Build history of the part. All positions in model axes, mm. A direction names the side the tool comes from. Give positions to 0.01 mm unless a question says otherwise; leave off trailing zeros. Order: outer loops, then holes, each group sorted by start corner. A loop starts at its lowest first (then second) coordinate and runs counter-clockwise, first axis right, second up. Notation, with made-up numbers: (88, -19.75) - (109, -19.75) arc R19 cw to (109, 15.25) - close; hole circle Ø9 at (44.5, 7.25). An arc over 180 degrees is marked (long way). Write each question's results on one line, items separated by ' | '. Start each with the question number.
1) Two-plate mould, pull along X, no slides. Class faces 1 (the face through (23, 97, -5)), 2 (the face through (-22, 98, -5)), 3 (the face through (1.774, 32.783, -1.775)): +X half, -X half, draft (parallel to the pull), parting line (faces both ways), or undercut.
2) Cut at B-B on x = 0. State how many separate pieces and enclosed holes the cut face has, plus the area to 3 significant figures.
3) Drill centre lines: line 1 along Y through (x, z) = (0, -6.75); line 2 along Y through (x, z) = (0, -2.1); line 3 along Z through (x, y) = (12.5, 6.25). Where is each one in solid material? Low to high. Write a range as from..to.
4) Cut at A-A on y = 60. List the corners of the cut face in (x, z), plus the area to 3 significant figures.
5) Cut at D-D on x = 12.5. List the corners of the cut face in (y, z).
6) Tool access for faces 4 (the face through (25, 38, -9)), 5 (the face through (0.716, 35.453, -6.845)), 6 (the face through (0, 54, -10)): list every direction of +Z, -Z, +X, -X, +Y, -Y with a clear straight run to the whole face (end or side of a thin tool).
7) Drop flat-ended pins along their axis: pin 1 Ø25 at (x, y) = (-1, 68) entering from -Z; pin 2 Ø9 at (x, y) = (0, 60) entering from +Z; pin 3 Ø9 at (x, z) = (6.5, -20.5) entering from +Y; pin 4 Ø5.5 at (x, y) = (0, 90) entering from +Z. Give the stop position or say it passes through.
8) Cut at C-C on z = -25. List the corners of the cut face in (x, y).
from build123d import *

# Parameters (mm, degrees)
EXTRUDE_2_DEPTH              = 25
HOLE_WIZARD_6_5_6_5_1_D      = 6.5
HOLE_WIZARD_M6_1_D           = 6.6
HOLE_WIZARD_M6_1_CBORE_D     = 11
HOLE_WIZARD_M6_1_CBORE_DEPTH = 6.4
CHAMFER_1_SIZE               = 5


with BuildPart() as part:
    # 草图2 → 拉伸-薄壁2 (new, symmetric)
    with BuildSketch(Plane(origin=(0, 0, 0), x_dir=(0, 0, -1), z_dir=(1, 0, 0))):
        Polygon((0, 100), (0, 0), (40, 0), (40, 10), (10, 10), (10, 100), align=None)
    extrude(amount=EXTRUDE_2_DEPTH, both=True)

    # Ø6.5 (6.5) 直径孔1 (through all)
    with Locations(Plane(origin=(0, 10, 0), x_dir=(1, 0, 0), z_dir=(0, 1, 0))):
        with Locations((-12.5, 25), (12.5, 25)):
            Hole(HOLE_WIZARD_6_5_6_5_1_D / 2)

    # M6 六角凹头螺钉的柱形沉头孔1 (through all)
    with Locations(Plane(origin=(0, 0, -10), x_dir=(-1, 0, 0), z_dir=(0, 0, -1))):
        with Locations((0, 90), (0, 60), (0, 30)):
            CounterBoreHole(HOLE_WIZARD_M6_1_D / 2, HOLE_WIZARD_M6_1_CBORE_D / 2, HOLE_WIZARD_M6_1_CBORE_DEPTH)

    # 倒角1
    chamfer_1_edges = [part.edges().sort_by_distance(p)[0] for p in [
        (25, 100, -5),
        (-25, 100, -5),
        (-25, 5, -40),
        (25, 5, -40),
    ]]
    chamfer(chamfer_1_edges, length=CHAMFER_1_SIZE)


solid = part.part
Results:
1) face 1: +X half | face 2: -X half | face 3: undercut
2) separate pieces: 4 | enclosed holes: 0 | area: 1,020 mm^2
3) line 1: 0..24.5, 35.5..54.5, 65.5..84.5, 95.5..100 | line 2: 0..26.7, 33.3..56.7, 63.3..86.7, 93.3..100 | line 3: -40..-28.25, -21.75..0
4) outline: (-25, -10) - (-5.5, -10) - (-5.5, -3.6) - (-3.3, -3.6) - (-3.3, 0) - (-25, 0) - close; (3.3, -3.6) - (5.5, -3.6) - (5.5, -10) - (25, -10) - (25, 0) - (3.3, 0) - close | area: 406 mm^2
5) outline: (0, -40) - (10, -40) - (10, -28.25) - (0, -28.25) - close; (0, -21.75) - (10, -21.75) - (10, -10) - (100, -10) - (100, 0) - (0, 0) - close
6) face 4: +Z, -Z, +X, +Y, -Y | face 5: -Z | face 6: -Z, +X, -X, +Y
7) pin 1: z = -10 | pin 2: z = 0 | pin 3: y = 10 | pin 4: through
8) outline: (-25, 0) - (-15.75, 0) - (-15.75, 10) - (-25, 10) - close; (-9.25, 0) - (9.25, 0) - (9.25, 10) - (-9.25, 10) - close; (15.75, 0) - (25, 0) - (25, 10) - (15.75, 10) - close
